Read the model definition and answer for the solid it produces. Units are mm, in the model's axes. A direction names the side the tool comes from. Coordinates: 2 decimals unless noted, no trailing zeros. Write each loop counter-clockwise with the first axis right and the second up, starting at its lowest first coordinate (ties: lowest second). Pieces come first, ordered by that corner, then holes. Notation, with made-up numbers: M -3,34 L 31,34 A15 ccw 31,53 Z; hole C 8,4.5 d1. An arc over 180 degrees is marked long. Write item = value, one per line.
from build123d import *

# Parameters (mm, degrees)
LEVER_PROFILE_SKETCH_R      = 21
HUB_BOSS_44MM_DEPTH         = 44
SLOTTED_ARM_BOSS_26MM_DEPTH = 26


with BuildPart() as part:
    # Lever Profile Sketch → Hub Boss 44mm (new body)
    with BuildSketch(Plane(origin=(0, 0, 0), x_dir=(1, 0, 0), z_dir=(0, 1, 0))):
        with Locations(Location((0, 0, 0), (0, 0, 270))):
            Circle(LEVER_PROFILE_SKETCH_R)
        with BuildLine():
            Line((11.618950039, 3), (14.618950039, 3))
            Line((14.618950039, 3), (14.618950039, -3))
            Line((14.618950039, -3), (11.618950039, -3))
            ThreePointArc((11.618950039, -3), (-12, 0), (11.618950039, 3))
        make_face(mode=Mode.SUBTRACT)
    extrude(amount=HUB_BOSS_44MM_DEPTH)

    # Sketch1_3 → Slotted Arm Boss 26mm (add)
    with BuildSketch(Plane(origin=(0, 0, 0), x_dir=(1, 0, 0), z_dir=(0, 1, 0))):
        with BuildLine():
            ThreePointArc((-20.784609691, -3), (-15.874507866, 13.747727085), (0, 21))
            Line((0, 21), (-80, 21))
            Line((-80, 21), (-80, 11))
            Line((-80, 11), (-60.656854249, 11))
            ThreePointArc((-60.656854249, 11), (-55, 15), (-49.343145751, 11))
            Line((-49.343145751, 11), (-40, 11))
            Line((-40, 11), (-40, 7))
            Line((-40, 7), (-49.343145751, 7))
            ThreePointArc((-49.343145751, 7), (-55, 3), (-60.656854249, 7))
            Line((-60.656854249, 7), (-80, 7))
            Line((-80, 7), (-80, -3))
            Line((-80, -3), (-20.784609691, -3))
        make_face()
    extrude(amount=SLOTTED_ARM_BOSS_26MM_DEPTH)


solid = part.part
Item 1: Flat-ended cylindrical pins translate along their axes: pin 1 (1 mm diameter, centred on y = 32.5, z = -11.5, fed in from +X); pin 2 (12 mm diameter, centred on x = -43, z = -9.5, fed in from +Y); pin 3 (1.5 mm diameter, centred on x = 12.5, y = 25, fed in from +Z); pin 4 (21.5 mm diameter, centred on x = 0, z = 0, fed in from +Y). Find the tip coordinate at first contact, or state that the pin passes through.
Worked answers:
pin_1 = 17.89
pin_2 = 26
pin_3 = 17.41
pin_4 = through
Item 2: Find section B-B (z = 1.5). Determine the outline of the cut face in (x, y).
Worked answers:
outline = M -80,0 L -11.91,0 L -11.91,44 L -20.95,44 L -20.95,26 L -80,26 Z; M 14.62,0 L 20.95,0 L 20.95,44 L 14.62,44 Z
Item 3: Consider line 1 along X through (y, z) = (26.5, 0); line 2 along X through (y, z) = (16, 0); line 3 along Z through (x, y) = (0, 29). Determine where each line is inside the solid, lowest interval first. Write a range as from..to.
Worked answers:
line_1 = -21..-12, 14.62..21
line_2 = -80..-12, 14.62..21
line_3 = -21..-12, 12..21
Item 4: Find section D-D (x = -5). Determine the outline of the cut face in (y, z), and give its area (3 significant figures).
Worked answers:
outline = M 0,-21 L 26,-21 L 26,-20.4 L 44,-20.4 L 44,-10.91 L 0,-10.91 Z; M 0,10.91 L 44,10.91 L 44,20.4 L 0,20.4 Z
area = 851 mm²
Item 5: Find section C-C (y = 31). Determine the outline of the cut face in (x, z).
Worked answers:
outline = C 0,0 d42; hole M 11.62,-3 L 14.62,-3 L 14.62,3 L 11.62,3 A12 ccw long Z
Item 6: For a pull along X with two mould halves and no side action, classify faces 4 (the face through (-80, 13, -2)), 5 (the face through (-39, 13, -21)), 6 (the face through (-55, 13, -3)) as released by +X, released by -X, zero draft, split by the parting line, or undercut.
Worked answers:
face_4 = released by -X
face_5 = zero draft
face_6 = undercut
Item 7: Find section A-A (x = -43). Determine the outline of the cut face in (y, z).
Worked answers:
outline = M 0,-21 L 26,-21 L 26,-11 L 0,-11 Z; M 0,-7 L 26,-7 L 26,3 L 0,3 Z
Item 8: Which of the six approach directions +Z, -Z, +X, -X, +Y, -Y give full straight-line access (tool end or side, diameter ignored) to faces 1 (the face through (-70, 13, -11)), 2 (the face through (-9, 44, 9)), 3 (the face through (13, 22, 3))?
Worked answers:
face_1 = -X, +Y, -Y
face_2 = +Z, -Z, +X, -X, +Y
face_3 = +Y, -Y
